from build123d import *


with BuildPart() as part:
    # Sketch1 → Revolve1 (revolve)
    with BuildSketch(Plane.XY, mode=Mode.PRIVATE) as revolve1_sk:
        Polygon((-50, 48.55), (-50, 50), (-44, 50), (-44, 44), (-50, 44), (-50, 46), (-45.5, 46), (-45.5, 48.55), align=None)
    revolve(revolve1_sk.sketch.rotate(Axis((0, 0, 0), (-1, 0, 0)), 90), axis=Axis((0, 0, 0), (-1, 0, 0)))


solid = part.part
Input: part model. Units: mm. Frame: model coordinates. A direction names the side the tool comes from. Round coordinates to 2 decimals unless told otherwise and drop trailing zeros. Write each loop counter-clockwise with the first axis right and the second up, starting at its lowest first coordinate (ties: lowest second). Pieces come first, ordered by that corner, then holes.
1) Contact query for flat-ended pins moving along their axis: P1, Ø1.5, axis at x = -48, y = 16, coming from the +Z side; P2, Ø2, axis at x = -48, y = 39.5, coming from the -Z side; P3, Ø1.5, axis at x = -47.5, y = 31, coming from the -Z side. Output: stop coordinate, or through.
2) Cut plane A-A (z = 0). Return the cut outline in (x, y), then the cut area to 4 significant figures.
3) Cut plane C-C (x = -46.6). Return the cut outline in (y, z).
4) Reachability of faces 4 (the flat face through (-44, 44.2, 0.2)), 5 (the cylindrical face through (-47.72, -45.61, 5.99)) from +Z, -Z, +X, -X, +Y, -Y: full face, straight path, thin tool, end or side. Return the list, or none.
5) Ray query, L1, parallel to Y at x = -48.9, z = 0; L2, parallel to Y at x = -48.35, z = -3.5; L3, parallel to Z at x = -46.05, y = 8.5. Return the intervals inside material, ascending.
6) Draft query along Y for faces 1 (the cylindrical face through (-46.96, -15.02, -47.69)), 2 (the cylindrical face through (-47.042, 42.954, 9.538)), 3 (the flat face through (-50, 41, 17)). Return one class per face: pulls with the +Y half, pulls with the -Y half, needs draft (parallel to the pull), parting line crosses it, or undercut.
Geometry says:
1. P1: stops at z = 47.62
1. P2: stops at z = -31.9
1. P3: stops at z = -39.81
2. outline: (-50, -50) - (-44, -50) - (-44, -44) - (-50, -44) - (-50, -46) - (-45.5, -46) - (-45.5, -48.55) - (-50, -48.55) - close; (-50, 44) - (-44, 44) - (-44, 50) - (-50, 50) - (-50, 48.55) - (-45.5, 48.55) - (-45.5, 46) - (-50, 46) - close
2. area: 49.05 mm2
3. outline: circle Ø100 at (0, 0); circle Ø92 at (0, 0); hole circle Ø97.1 at (0, 0); hole circle Ø88 at (0, 0)
4. face 4: +Z, -Z, +X, +Y, -Y
4. face 5: -X
5. L1: y = -50 to -48.55, -46 to -44, 44 to 46, 48.55 to 50
5. L2: y = -49.88 to -48.42, -45.87 to -43.86, 43.86 to 45.87, 48.42 to 49.88
5. L3: z = -49.27 to -47.8, -45.21 to -43.17, 43.17 to 45.21, 47.8 to 49.27
6. face 1: parting line crosses it
6. face 2: undercut
6. face 3: needs draft
